Here's how the part is built. I have some questions about the finished solid (model axes, mm). A direction names the side the tool comes from. Give positions to 0.01 mm unless a question says otherwise; leave off trailing zeros. Order: outer loops, then holes, each group sorted by start corner. A loop starts at its lowest first (then second) coordinate and runs counter-clockwise, first axis right, second up. Notation, with made-up numbers: (-39.75, -19) - (18.25, -19) arc R24 ccw to (18.25, -3) - close; hole circle Ø5 at (54.25, -37.75). An arc over 180 degrees is marked (long way). One line per question, with ' | ' between items.
from build123d import *

# Parameters (mm, degrees)
BOSS_EXTRUDE1_DEPTH = 20
SKETCH2_R           = 5
BOSS_EXTRUDE2_DEPTH = 22.5
SKETCH4_R           = 5
CUT_EXTRUDE1_DEPTH  = 0.5
CIRPATTERN1_COUNT   = 3


with BuildPart() as part:
    # Sketch1 → Boss-Extrude1 (new body)
    with BuildSketch(Plane.XY):
        Polygon((50, 0), (25, 43.301270189), (-25, 43.301270189), (-50, 0), (-25, -43.301270189), (25, -43.301270189), align=None)
    extrude(amount=BOSS_EXTRUDE1_DEPTH)

    # Sketch2 → Boss-Extrude2 (add, symmetric)
    with BuildSketch(Plane(origin=(0, 0, 0), x_dir=(0, 0, -1), z_dir=(1, 0, 0))):
        with BuildLine():
            Line((-20, 43.301270189), (-23.46513086, 55.465896517))
            ThreePointArc((-23.46513086, 55.465896517), (-10.001520995, 73.301270167), (3.464086976, 55.467405029))
            Line((3.464086976, 55.467405029), (0, 43.301270189))
            Line((0, 43.301270189), (-20, 43.301270189))
        make_face()
        with Locations(Location((-10.000736748, 59.301270189, 0), (0, 0, 180))):
            Circle(SKETCH2_R, mode=Mode.SUBTRACT)
    boss_extrude2 = extrude(amount=BOSS_EXTRUDE2_DEPTH, both=True)

    # Sketch4 → Cut-Extrude1 (cut)
    with BuildSketch(Plane(origin=(0, 0, 0), x_dir=(-1, 0, 0), z_dir=(0, 0, -1))):
        Circle(SKETCH4_R)
    extrude(amount=-CUT_EXTRUDE1_DEPTH, mode=Mode.SUBTRACT)

    # CirPattern1: Boss-Extrude2 ×3 about axis
    cirpattern1_axis = Axis((0, 0, 0), (0, 0, 1))
    for i in range(1, CIRPATTERN1_COUNT):
        add(boss_extrude2.rotate(cirpattern1_axis, i * 360 / CIRPATTERN1_COUNT))


solid = part.part
1) Thinking about a two-plate mould opening in X: for faces 1 (the face through (-46.91, -27.44, 9.35)), 2 (the face through (-37.3, 22, 9.9)), 3 (the face through (0.315, 49.47, -1.756)), which applies, +X half, -X half, draft (parallel to the pull), parting line (faces both ways), or undercut?
Model answer:
face 1: undercut | face 2: -X half | face 3: draft
2) I want a section at A-A (x = 0). List the corners of the cut face in (y, z) for me, plus the area to 3 significant figures.
Model answer:
outline: (-43.3, 0) - (-5, 0) - (-5, 0.5) - (5, 0.5) - (5, 0) - (43.3, 0) - (55.47, -3.46) arc R14 ccw (long way) to (55.47, 23.47) - (43.3, 20) - (-43.3, 20) - close; hole circle Ø10 at (59.3, 10) | area: 2,350 mm2
3) I want a section at C-C (x = -30). List the corners of the cut face in (y, z) for me, plus the area to 3 significant figures.
Model answer:
outline: (-43.3, -1.23) - (-34.64, 0) - (34.64, 0) - (34.64, 20) - (-34.64, 20) - (-43.3, 21.23) - close | area: 1,570 mm2
4) I'm going to push flat-ended pins straight in: P1, Ø5, axis at x = 33.5, y = -33, coming from the -Z side; P2, Ø6, axis at x = -33.5, z = 14, coming from the -Y side; P3, Ø5, axis at x = 48.5, z = 16.5, coming from the -Y side. Where does each tip first touch, or does it pass through?
Model answer:
P1: stops at z = -1.34 | P2: stops at y = -47.05 | P3: stops at y = -55.41
5) I want a section at B-B (y = 10.5). List the corners of the cut face in (x, z) for me.
Model answer:
outline: (-43.94, 0) - (43.94, 0) - (43.94, 20) - (-43.94, 20) - close
6) Please list where these lines run through material, in increasing order: L1, parallel to Y at x = 2.5, z = 10; L2, parallel to X at y = -15, z = 9.5; L3, parallel to Z at x = -53.5, y = -31.5.
Model answer:
L1: y = -43.3 to 54.3, 64.3 to 73.3 | L2: x = -70.98 to -65.56, -54.07 to 54.07, 65.56 to 70.98 | L3: z = -3.72 to 5.85, 14.16 to 23.72
7) On a 3-axis mill with a long thin cutter (end or side, diameter ignored), from which of +Z, -Z, +X, -X, +Y, -Y can I reach the whole of each face in a straight line? I mean faces 4 (the face through (0, -43.301, 10)), 5 (the face through (-1, 1, 20)), 6 (the face through (42.684, -25.008, -1.756)). Say none if no direction works.
Model answer:
face 4: +Z, -Z, -Y | face 5: +Z | face 6: -Z, +Y
